Source: three-view drawing plus pictorial views. Frame: mm from the lowest corner of the part. A direction names the side the tool comes from. Round coordinates to 2 decimals unless told otherwise and drop trailing zeros. Loops run counter-clockwise (first coordinate to the right, second up) from the corner with the lowest first, then second, coordinate; pieces in that order, holes last. Notation, with made-up numbers: (80, 75.25) -> (136, 75.25) arc R25 ccw to (136, 92.25) -> close; hole circle Ø10 at (68, 28.25). An arc over 180 degrees is marked (long way). Answer in a Markdown table with one row per item. Add a question column.
Q1. Section C-C, the plane x = 0.65. Give the number of separate pieces and of enclosed holes in the cut face.
Q2. Ray query, L1, parallel to Z at x = 0.35, y = 3.25 (1 decimal); L2, parallel to Y at x = 0.2, z = 8.1 (1 decimal); L3, parallel to Y at x = 0.85, z = 4 (1 decimal). Return the intervals inside material, ascending. Write a range as from..to.
Q3. Reachability of the marked faces 1 and 2 from +Z, -Z, +X, -X, +Y, -Y: full face, straight path, thin tool, end or side. Return the list, or none.
Q4. Mould query, pull axis Y, two halves, no side actions, for the marked faces 3, 4 and 5. Classes: pulls with the +Y half, pulls with the -Y half, needs draft (parallel to the pull), parting line crosses it, or undercut.
Q5. Section A-A, the plane y = 6. Output: boundary loops of the cut face in (x, z).
Q6. Section D-D, the plane y = 7.75. Output: boundary loops of the cut face in (x, z).
Q7. Section B-B, the plane z = 8.5. Output: boundary loops of the cut face in (x, y).
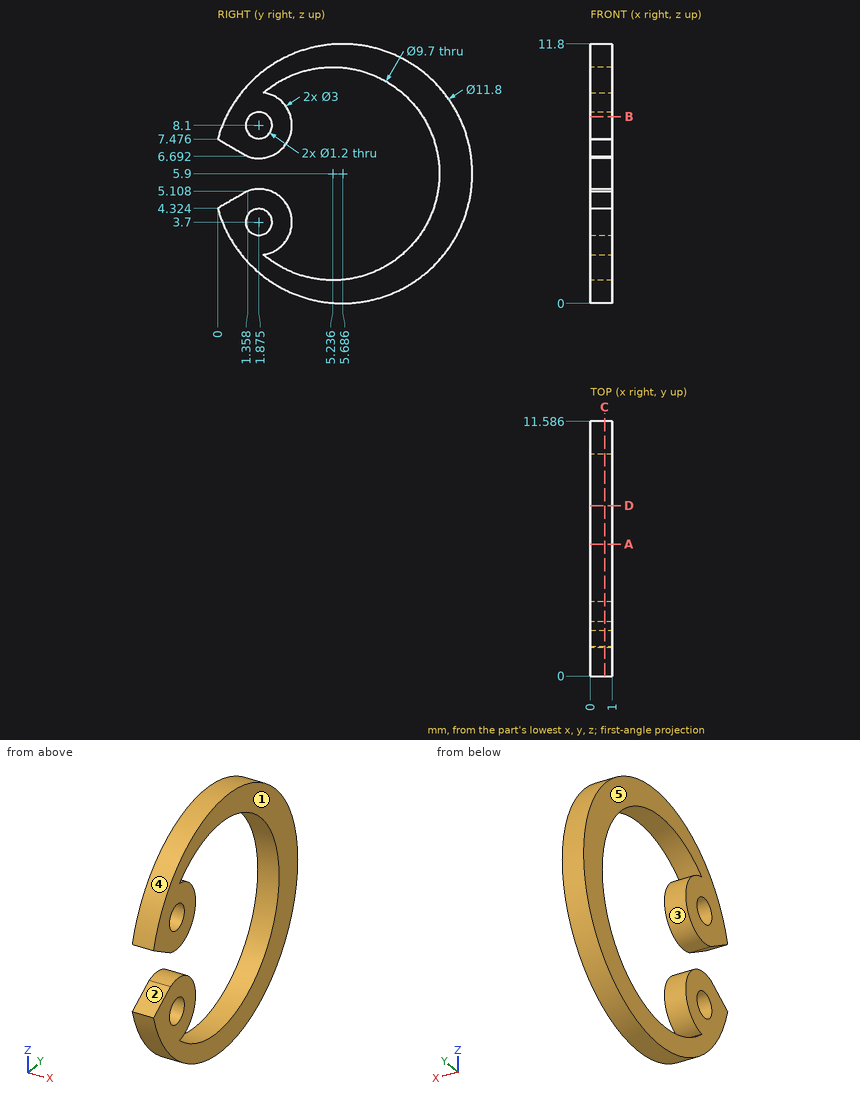
Answer block:
| question | item | result |
|---|---|---|
| 1 | separate pieces | 1 |
| 1 | enclosed holes | 2 |
| 2 | L1 | 0.5..1.5, 3.1..4.3, 7.5..8.7, 10.3..11.3 |
| 2 | L2 | 0.2..1.3, 2.5..3.4, 9.6..11.2 |
| 2 | L3 | 0.1..1.4, 2.4..3.3, 9.7..11.3 |
| 3 | face 1 | +Z, -Z, +X, +Y, -Y |
| 3 | face 2 | +X, -X, -Y |
| 4 | face 3 | undercut |
| 4 | face 4 | parting line crosses it |
| 4 | face 5 | needs draft |
| 5 | outline | (0, 0.01) -> (1, 0.01) -> (1, 1.11) -> (0, 1.11) -> close; (0, 10.69) -> (1, 10.69) -> (1, 11.79) -> (0, 11.79) -> close |
| 6 | outline | (0, 0.37) -> (1, 0.37) -> (1, 1.75) -> (0, 1.75) -> close; (0, 10.05) -> (1, 10.05) -> (1, 11.43) -> (0, 11.43) -> close |
| 7 | outline | (0, 0.39) -> (1, 0.39) -> (1, 1.43) -> (0, 1.43) -> close; (0, 2.32) -> (1, 2.32) -> (1, 3.32) -> (0, 3.32) -> close; (0, 9.33) -> (1, 9.33) -> (1, 10.98) -> (0, 10.98) -> close |
